For this review, take the finished solid that the model builds, in its own axes (mm). Round coordinates to 2 decimals unless told otherwise and drop trailing zeros. Write each loop counter-clockwise with the first axis right and the second up, starting at its lowest first coordinate (ties: lowest second). Pieces come first, ordered by that corner, then holes. Notation, with made-up numbers: M 21,-8 L 33,-8 A16 cw 33,10 Z; hole C -12,7 d3. An arc over 180 degrees is marked long. Answer in a Markdown table with one row per item.
```python
from build123d import *

# Parameters (mm, degrees)
SKETCH1_W                 = 150
SKETCH1_H                 = 200
BOSS_EXTRUDE1_DEPTH       = 25
F_3_4_10_THREADED_HOLE1_D = 16.66748


with BuildPart() as part:
    # Sketch1 → Boss-Extrude1 (new body)
    with BuildSketch(Plane.XY):
        with Locations((75, 100)):
            Rectangle(SKETCH1_W, SKETCH1_H)
    extrude(amount=BOSS_EXTRUDE1_DEPTH)

    # 3/4-10 Threaded hole1 (through all)
    with Locations(Plane(origin=(25, 125, 25), x_dir=(1, 0, 0), z_dir=(0, 0, 1))):
        with Locations((0, 0), (100, 0), (0, -100), (100, -100)):
            Hole(F_3_4_10_THREADED_HOLE1_D / 2)


solid = part.part
```
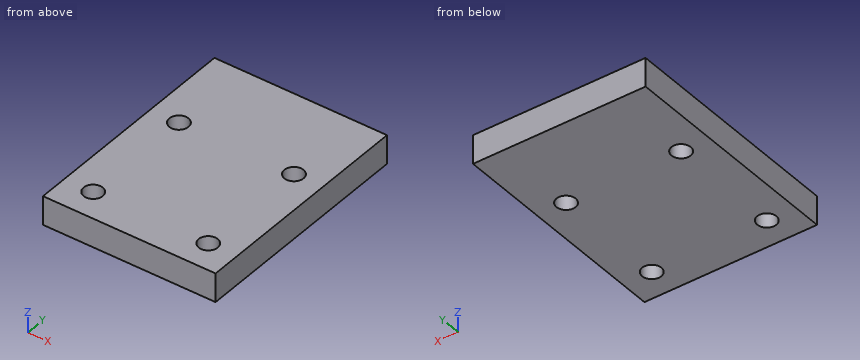
Q1. Take a section at C-C (z = 15.25). State the section outline as (x, y) points.
Found:
| item | result |
|---|---|
| outline | M 0,0 L 150,0 L 150,200 L 0,200 Z; hole C 25,25 d16.67; hole C 25,125 d16.67; hole C 125,25 d16.67; hole C 125,125 d16.67 |
Q2. Insertion check: P1, Ø15, axis at x = 25, y = 125, coming from the +Z side. The pin has a flat end and moves straight along its axis. Give the tip position at first contact, or say it passes through.
Found:
| item | result |
|---|---|
| P1 | through |
Q3. Take a section at A-A (y = 25). State the section outline as (x, z) points, then the cut area to 3 significant figures.
Found:
| item | result |
|---|---|
| outline | M 0,0 L 16.67,0 L 16.67,25 L 0,25 Z; M 33.33,0 L 116.67,0 L 116.67,25 L 33.33,25 Z; M 133.33,0 L 150,0 L 150,25 L 133.33,25 Z |
| area | 2,920 mm² |
Q4. For probe 1 along Y at (x, z) = (125, 15); probe 2 along Y at (x, z) = (17.5, 14.25); probe 3 along X at (y, z) = (22.5, 20.25), list the stretches that pass through material, from the lowest coordinate up.
Found:
| item | result |
|---|---|
| probe 1 | 0 to 16.67, 33.33 to 116.67, 133.33 to 200 |
| probe 2 | 0 to 21.37, 28.63 to 121.37, 128.63 to 200 |
| probe 3 | 0 to 17.05, 32.95 to 117.05, 132.95 to 150 |
Q5. Take a section at B-B (x = 25). State the section outline as (y, z) points, then the cut area to 3 significant figures.
Found:
| item | result |
|---|---|
| outline | M 0,0 L 16.67,0 L 16.67,25 L 0,25 Z; M 33.33,0 L 116.67,0 L 116.67,25 L 33.33,25 Z; M 133.33,0 L 200,0 L 200,25 L 133.33,25 Z |
| area | 4,170 mm² |
